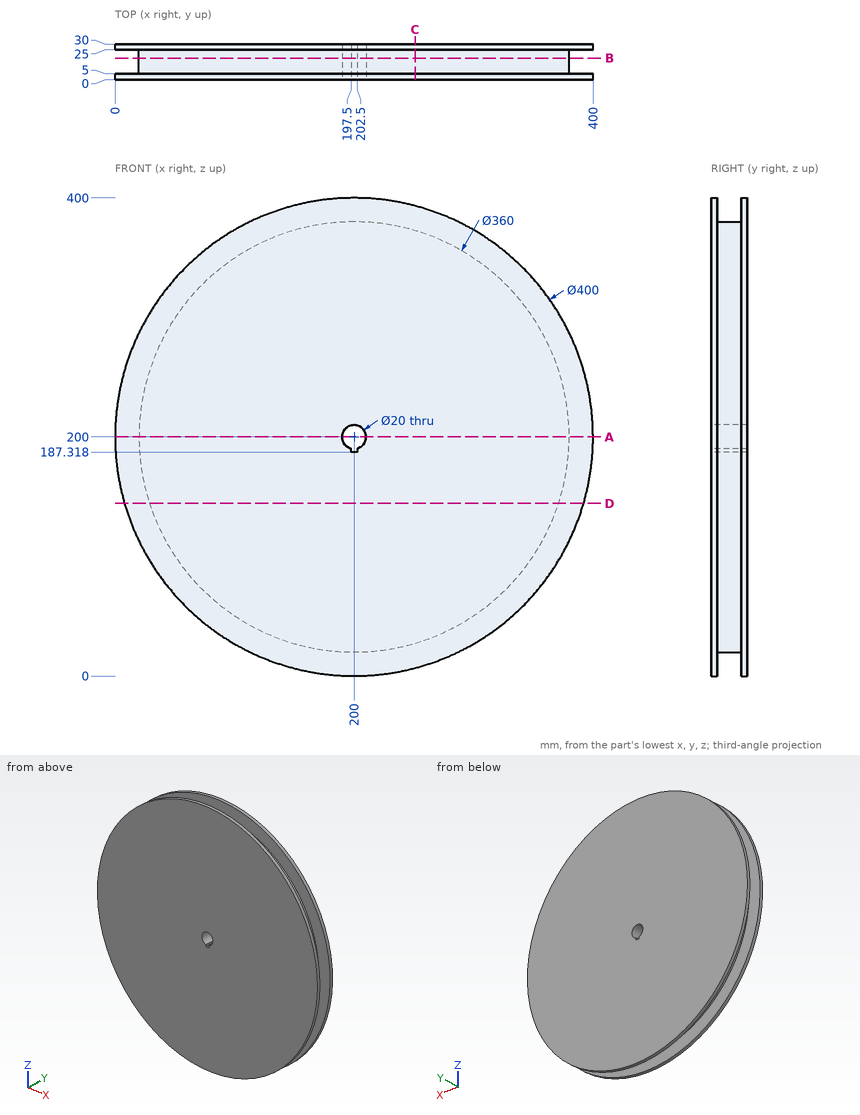
Geometry: see drawing. Coordinates: mm, zero at the bounding-box minimum. Give positions to 0.01 mm unless a question says otherwise; leave off trailing zeros. Order: outer loops, then holes, each group sorted by start corner. A loop starts at its lowest first (then second) coordinate and runs counter-clockwise, first axis right, second up.
Q1. Contact query for flat-ended pins moving along their axis: pin 1 Ø1.5 at (y, z) = (3.5, 287) entering from -X; pin 2 Ø1.5 at (x, y) = (199.5, 10.5) entering from +Z; pin 3 Ø1 at (x, z) = (101, 155) entering from -Y; pin 4 Ø1 at (x, y) = (350.5, 17.5) entering from -Z. Output: stop coordinate, or through.
Checked values:
pin 1: stops at x = 19.55
pin 2: stops at z = 380
pin 3: stops at y = 0
pin 4: stops at z = 100.5
Q2. Section C-C on x = 251. Output: boundary loops of the cut face in (y, z).
Checked values:
outline: (0, 6.61) - (5, 6.61) - (5, 27.38) - (25, 27.38) - (25, 6.61) - (30, 6.61) - (30, 393.39) - (25, 393.39) - (25, 372.62) - (5, 372.62) - (5, 393.39) - (0, 393.39) - close
Q3. Ray query, probe 1 along Y at (x, z) = (370, 262); probe 2 along X at (y, z) = (10.75, 200); probe 3 along X at (y, z) = (4, 324). Return the intervals inside material, ascending.
Checked values:
probe 1: y = 0 to 5, 25 to 30
probe 2: x = 20 to 190, 210 to 380
probe 3: x = 43.08 to 356.92
Q4. Section A-A on z = 200. Output: boundary loops of the cut face in (x, y), and give its area (3 significant figures).
Checked values:
outline: (0, 0) - (190, 0) - (190, 30) - (0, 30) - (0, 25) - (20, 25) - (20, 5) - (0, 5) - close; (210, 0) - (400, 0) - (400, 5) - (380, 5) - (380, 25) - (400, 25) - (400, 30) - (210, 30) - close
area: 10,600 mm2
Q5. Section B-B on y = 18.25. Output: boundary loops of the cut face in (x, z), and give its area (3 significant figures).
Checked values:
outline: circle Ø360 at (200, 200); hole (197.5, 187.32) - (202.5, 187.32) - (202.5, 190.32) arc R10 ccw (long way) to (197.5, 190.32) - close
area: 101,000 mm2
Q6. Section D-D on z = 144.5. Output: boundary loops of the cut face in (x, y) (1 decimal), and give its area (3 significant figures).
Checked values:
outline: (7.9, 0) - (392.1, 0) - (392.1, 5) - (371.2, 5) - (371.2, 25) - (392.1, 25) - (392.1, 30) - (7.9, 30) - (7.9, 25) - (28.8, 25) - (28.8, 5) - (7.9, 5) - close
area: 10,700 mm2
